Geometry: final body of the model. Coordinates: model frame, mm. Face numbers are marked on the shaded views. Round coordinates to 2 decimals unless told otherwise and drop trailing zeros. Loops run counter-clockwise (first coordinate to the right, second up) from the corner with the lowest first, then second, coordinate; pieces in that order, holes last. Notation, with made-up numbers: (-1.5, 12.5) - (4.5, 12.5) arc R7 ccw to (4.5, 24.5) - close; hole circle Ø10 at (25.5, 20.5). An arc over 180 degrees is marked (long way). Return JSON: item names as keys, results as strings. Group by question number.
1. Section B-B on z = 0. Return loops of the section in (x, y) (3 decimals), and give its area (3 significant figures).
2. Material intervals for probe 1 along X at (y, z) = (0.85, 0); probe 2 along Y at (x, z) = (40.5, -16); probe 3 along Z at (x, y) = (-39.5, 1.1), sorted ascending.
3. First-contact query: pin 1 Ø1.5 at (y, z) = (2, 48) entering from +X; pin 2 Ø2 at (x, y) = (12, 2.5) entering from -Z; pin 3 Ø3 at (x, y) = (7.5, 2) entering from -Z; pin 4 Ø2 at (x, z) = (-7, -30.5) entering from +Y. Flat tips, straight axial feed; report the tip coordinate or a pass-through.
4. Draft query along X for the marked faces 1, 2, 3 and 4. Return one class per face: +X half, -X half, draft (parallel to the pull), parting line (faces both ways), or undercut.
5. Section A-A on x = -18. Return loops of the section in (y, z) (3 decimals), and give its area (3 significant figures).
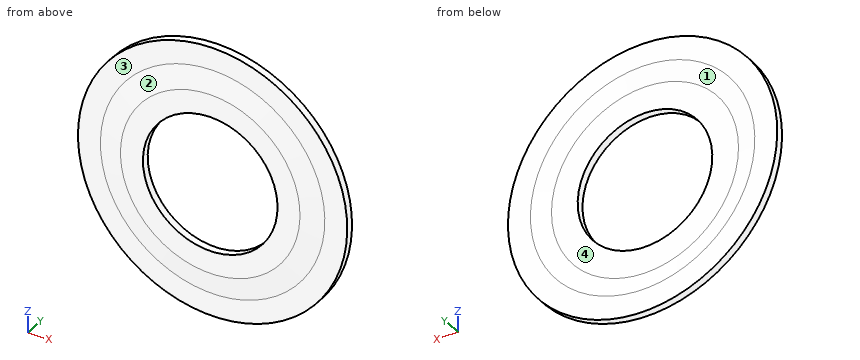
from build123d import *

# Parameters (mm, degrees)
SCALE_1_SCALE = 1.875


with BuildPart() as part:
    # Sketch1 → Revolve1 (revolve)
    with BuildSketch(Plane.XY, mode=Mode.PRIVATE) as revolve1_sk:
        Polygon((0, 0), (0, 2), (7, 2), (12, 2.997347898), (18, 2.997347898), (18, 1), (12, 1), (6, 0), align=None)
    revolve(revolve1_sk.sketch.rotate(Axis((-18, 6.77671814, 0), (0, -1, 0)), 90), axis=Axis((-18, 6.77671814, 0), (0, -1, 0)))


with BuildPart() as part_1:
    # Scale 1: scaled about (-18, 1.56874625, 0)
    add(part.part.scale(SCALE_1_SCALE).moved(Location((15.75, -1.372652969, 0))))


solid = part_1.part
Taken from the geometry:
{
 "1": {"outline": "(-85.5, 0.502) - (-74.25, 0.502) - (-63, -1.373) - (-51.75, -1.373) - (-51.75, 2.377) - (-64.875, 2.377) - (-74.25, 4.247) - (-85.5, 4.247) - close; (15.75, -1.373) - (27, -1.373) - (38.25, 0.502) - (49.5, 0.502) - (49.5, 4.247) - (38.25, 4.247) - (28.875, 2.377) - (15.75, 2.377) - close", "area": "249 mm2"},
 "2": {"probe 1": "-85.5 to -51.75, 15.75 to 49.5", "probe 2": "0.5 to 4.25", "probe 3": "-63.98 to -26.02, 26.02 to 63.98"},
 "3": {"pin 1": "x = 30.2", "pin 2": "z = -60.95", "pin 3": "z = -63.09", "pin 4": "through"},
 "4": {"face 1": "undercut", "face 2": "parting line", "face 3": "draft", "face 4": "undercut"},
 "5": {"outline": "(-1.373, -45) - (0.502, -56.25) - (0.502, -67.5) - (4.247, -67.5) - (4.247, -56.25) - (2.377, -46.875) - (2.377, -33.75) - (-1.373, -33.75) - close; (-1.373, 33.75) - (2.377, 33.75) - (2.377, 46.875) - (4.247, 56.25) - (4.247, 67.5) - (0.502, 67.5) - (0.502, 56.25) - (-1.373, 45) - close", "area": "249 mm2"}
}
